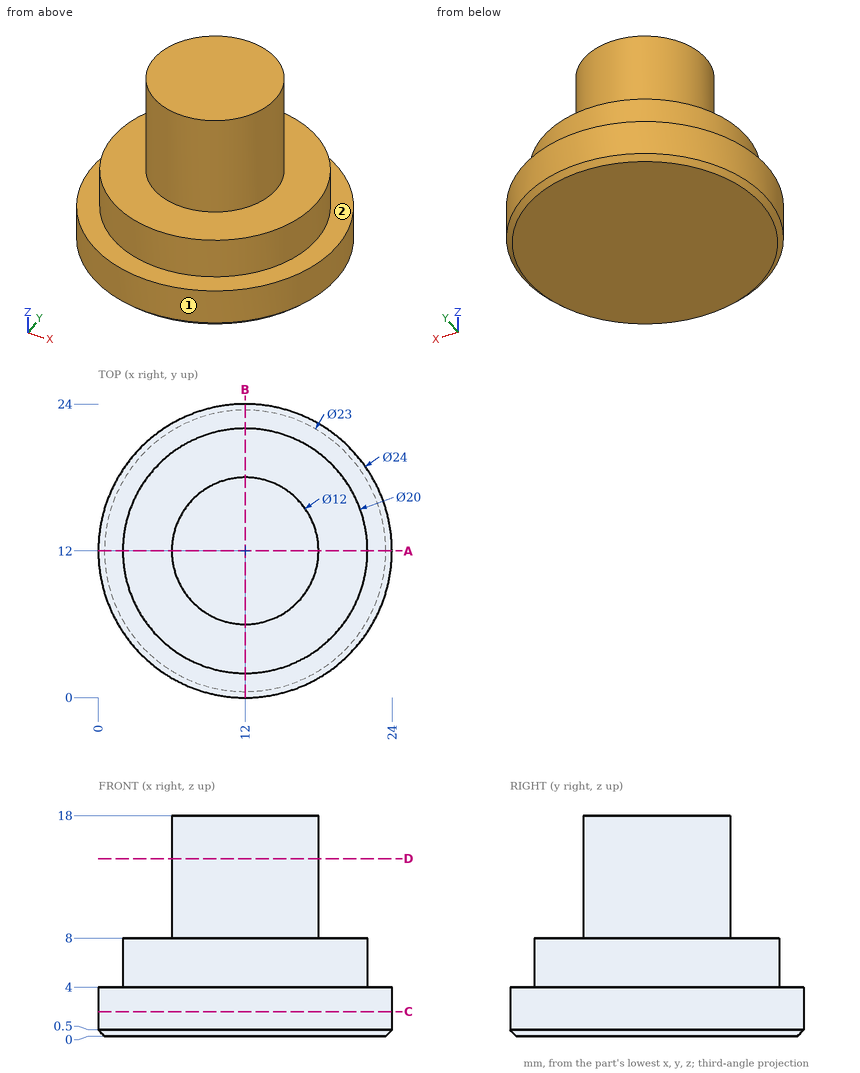
Check sheet for the drawn part. Datum: minimum x, y, z corner. Units: mm. A direction names the side the tool comes from. Round coordinates to 2 decimals unless told otherwise and drop trailing zeros. Write each loop counter-clockwise with the first axis right and the second up, starting at its lowest first coordinate (ties: lowest second). Pieces come first, ordered by that corner, then holes. Notation, with made-up numbers: (2.5, -25) -> (55.5, -25) arc R11 ccw to (55.5, -18) -> close; hole circle Ø11 at (44.25, -28.75). An arc over 180 degrees is marked (long way). Write each question's results on one line, items separated by ' | '.
Q1. Sectioned sample at C-C, the plane z = 2. Record the boundary of the cut face in (x, y), and give its area (3 significant figures).
Derived:
outline: circle Ø24 at (12, 12) | area: 452 mm²
Q2. Thickness scan on probe 1 along Z at (x, y) = (5, 9); probe 2 along Y at (x, z) = (12.25, 12.75); probe 3 along Z at (x, y) = (2.5, 7.75). Record the ranges inside material, lowest first.
Derived:
probe 1: z = 0 to 8 | probe 2: y = 6.01 to 17.99 | probe 3: z = 0 to 4
Q3. Access from +Z, -Z, +X, -X, +Y, -Y to the whole of each face (thin tool, end or side, straight path). Record for the marked faces 1 and 2.
Derived:
face 1: +Z, -Z | face 2: +Z
Q4. Go/stop test with flat-tipped pins: pin 1 Ø1.5 at (y, z) = (9, 5.5) entering from +X; pin 2 Ø6 at (y, z) = (18, 3) entering from -X; pin 3 Ø6 at (x, z) = (5.5, 2.5) entering from +Y. Record where each tip stops, or that it passes through.
Derived:
pin 1: stops at x = 21.74 | pin 2: stops at x = 0.38 | pin 3: stops at y = 23.48
Q5. Sectioned sample at A-A, the plane y = 12. Record the boundary of the cut face in (x, z), and give its area (3 significant figures).
Derived:
outline: (0, 0.5) -> (0.5, 0) -> (23.5, 0) -> (24, 0.5) -> (24, 4) -> (22, 4) -> (22, 8) -> (18, 8) -> (18, 18) -> (6, 18) -> (6, 8) -> (2, 8) -> (2, 4) -> (0, 4) -> close | area: 296 mm²
Q6. Sectioned sample at D-D, the plane z = 14.5. Record the boundary of the cut face in (x, y), and give its area (3 significant figures).
Derived:
outline: circle Ø12 at (12, 12) | area: 113 mm²
